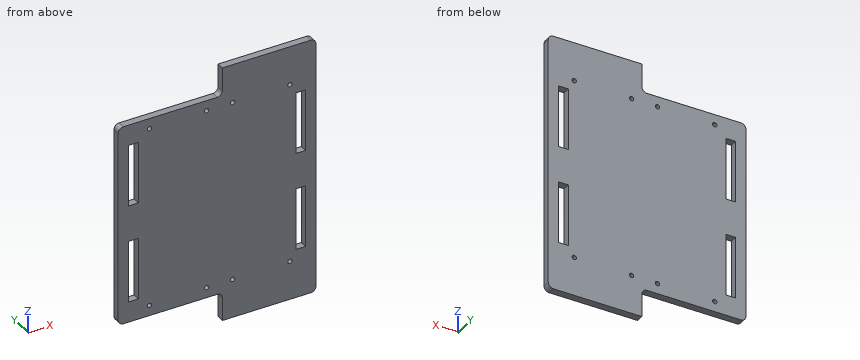
```python
from build123d import *

# Parameters (mm, degrees)
SKETCH1_W                   = 380
SKETCH1_H                   = 500
BOSS_EXTRUDE1_DEPTH         = 14
SKETCH2_W                   = 200
SKETCH2_H                   = 55
CUT_EXTRUDE1_DEPTH          = 14
FILLET1_R                   = 10
SKETCH3_W                   = 18.5
SKETCH3_H                   = 120
CUT_EXTRUDE2_DEPTH          = 20
M10_TAPPED_HOLE1_AT_2_COUNT = 2
M10_TAPPED_HOLE1_AT_2_PITCH = 110
M10_TAPPED_HOLE1_AT_3_COUNT = 2
M10_TAPPED_HOLE1_AT_3_PITCH = 366.878726557
M10_TAPPED_HOLE1_AT_4_COUNT = 2
M10_TAPPED_HOLE1_AT_4_PITCH = 350
LPATTERN1_COUNT             = 2
LPATTERN1_PITCH             = 160
FILLET2_R                   = 10


with BuildPart() as part:
    # Sketch1 → Boss-Extrude1 (new body)
    with BuildSketch(Plane(origin=(0, 0, 0), x_dir=(1, 0, 0), z_dir=(0, 1, 0))):
        Rectangle(SKETCH1_W, SKETCH1_H)
    extrude(amount=BOSS_EXTRUDE1_DEPTH)

    # Sketch2 → Cut-Extrude1 (cut)
    with BuildSketch(Plane(origin=(0, 14, 0), x_dir=(1, 0, 0), z_dir=(0, 1, 0))):
        with Locations((-90, 222.5)):
            Rectangle(SKETCH2_W, SKETCH2_H)
        with Locations((-90, -222.5)):
            Rectangle(SKETCH2_W, SKETCH2_H)
    extrude(amount=-CUT_EXTRUDE1_DEPTH, mode=Mode.SUBTRACT)

    # Fillet1
    fillet1_edges = [part.edges().sort_by_distance(p)[0] for p in [
        (10, 7, -195),
        (10, 7, 195),
    ]]
    fillet(fillet1_edges, radius=FILLET1_R)

    # Sketch3 → Cut-Extrude2 (cut)
    with BuildSketch(Plane(origin=(0, 14, 0), x_dir=(1, 0, 0), z_dir=(0, 1, 0))):
        with Locations((160.75, 95)):
            Rectangle(SKETCH3_W, SKETCH3_H)
        with Locations((160.75, -95)):
            Rectangle(SKETCH3_W, SKETCH3_H)
        with Locations((-160.75, -95)):
            Rectangle(SKETCH3_W, SKETCH3_H)
        with Locations((-160.75, 95)):
            Rectangle(SKETCH3_W, SKETCH3_H)
    extrude(amount=-CUT_EXTRUDE2_DEPTH, mode=Mode.SUBTRACT)

    # Sketch5 → M10 Tapped Hole1 (revolve, cut)
    with BuildSketch(Plane(origin=(30, 14, 175), x_dir=(0, 0, 1), z_dir=(1, 0, 0))):
        Polygon((0, 0), (0, 55.553657631), (4.25, 53), (4.25, 0), align=None)
    m10_tapped_hole1 = revolve(axis=Axis((30, 20.35, 175), (0, -1, 0)), mode=Mode.SUBTRACT)

    # M10 Tapped Hole1 at 2: M10 Tapped Hole1 ×2
    with Locations(*[(i * M10_TAPPED_HOLE1_AT_2_PITCH, 0, 0) for i in range(1, M10_TAPPED_HOLE1_AT_2_COUNT)]):
        add(m10_tapped_hole1, mode=Mode.SUBTRACT)

    # M10 Tapped Hole1 at 3: M10 Tapped Hole1 ×2
    with Locations(*[Vector(0.29982659674039447, 0, -0.9539937169012556) * (i * M10_TAPPED_HOLE1_AT_3_PITCH) for i in range(1, M10_TAPPED_HOLE1_AT_3_COUNT)]):
        add(m10_tapped_hole1, mode=Mode.SUBTRACT)

    # M10 Tapped Hole1 at 4: M10 Tapped Hole1 ×2
    with Locations(*[(0, 0, -i * M10_TAPPED_HOLE1_AT_4_PITCH) for i in range(1, M10_TAPPED_HOLE1_AT_4_COUNT)]):
        add(m10_tapped_hole1, mode=Mode.SUBTRACT)

    # LPattern1: M10 Tapped Hole1 ×2
    with Locations(*[(-i * LPATTERN1_PITCH, 0, 0) for i in range(1, LPATTERN1_COUNT)]):
        add(m10_tapped_hole1, mode=Mode.SUBTRACT)

    # LPattern1 copy 1 sketch → LPattern1 copy 1 (revolve, cut)
    with BuildSketch(Plane(origin=(-20, 14, 175), x_dir=(0, 0, 1), z_dir=(1, 0, 0))):
        Polygon((0, 0), (0, 55.553657631), (4.25, 53), (4.25, 0), align=None)
    revolve(axis=Axis((-20, 20.35, 175), (0, -1, 0)), mode=Mode.SUBTRACT)

    # LPattern1 copy 2 sketch → LPattern1 copy 2 (revolve, cut)
    with BuildSketch(Plane(origin=(-20, 14, -175), x_dir=(0, 0, 1), z_dir=(1, 0, 0))):
        Polygon((0, 0), (0, 55.553657631), (4.25, 53), (4.25, 0), align=None)
    revolve(axis=Axis((-20, 20.35, -175), (0, -1, 0)), mode=Mode.SUBTRACT)

    # LPattern1 copy 3 sketch → LPattern1 copy 3 (revolve, cut)
    with BuildSketch(Plane(origin=(-130, 14, -175), x_dir=(0, 0, 1), z_dir=(1, 0, 0))):
        Polygon((0, 0), (0, 55.553657631), (4.25, 53), (4.25, 0), align=None)
    revolve(axis=Axis((-130, 20.35, -175), (0, -1, 0)), mode=Mode.SUBTRACT)

    # Fillet2
    fillet2_edges = [part.edges().sort_by_distance(p)[0] for p in [
        (-190, 7, -195),
        (-190, 7, 195),
        (190, 7, 250),
        (190, 7, -250),
    ]]
    fillet(fillet2_edges, radius=FILLET2_R)


solid = part.part
```
Design review of the part built by this model. Coordinates are the model's own, in mm. Give positions to 0.01 mm unless a question says otherwise; leave off trailing zeros. Loops run counter-clockwise (first coordinate to the right, second up) from the corner with the lowest first, then second, coordinate; pieces in that order, holes last. Notation, with made-up numbers: (19, -14.5) -> (54, -14.5) arc R13 ccw to (54, -2.5) -> close; hole circle Ø10 at (66.5, -31.5). An arc over 180 degrees is marked (long way). One line per item, written item: value.
Q1. For L1, parallel to X at y = 9.5, z = -175; L2, parallel to X at y = 2, z = 38; L3, parallel to Z at x = -130, y = 4, list the stretches that pass through material, from the lowest coordinate up.
Numbers:
L1: x = -190 to -134.25, -125.75 to -24.25, -15.75 to 25.75, 34.25 to 135.75, 144.25 to 190
L2: x = -190 to -170, -151.5 to 151.5, 170 to 190
L3: z = -195 to -179.25, -170.75 to 170.75, 179.25 to 195
Q2. We need section B-B on y = 4.75. Give the number of separate pieces and of enclosed holes in the cut face, and give its area (3 significant figures).
Numbers:
separate pieces: 1
enclosed holes: 12
area: 159,000 mm^2
Q3. For pin 1 Ø7 at (x, z) = (140, 175) entering from +Y; pin 2 Ø4 at (y, z) = (4.5, -233) entering from -X; pin 3 Ø4 at (x, y) = (7, 7.5) entering from +Z; pin 4 Ø4 at (x, y) = (-159.5, 6.5) entering from +Z, all flat-tipped, find the tip position at first contact; note any pin that passes through.
Numbers:
pin 1: passes through
pin 2: stops at x = 10
pin 3: stops at z = 200.64
pin 4: stops at z = 195
Q4. We need section A-A on z = 56.5. Give the boundary of the cut face in (x, y).
Numbers:
outline: (-190, 0) -> (-170, 0) -> (-170, 14) -> (-190, 14) -> close; (-151.5, 0) -> (151.5, 0) -> (151.5, 14) -> (-151.5, 14) -> close; (170, 0) -> (190, 0) -> (190, 14) -> (170, 14) -> close
